Geometry: final body of the model. Coordinates: model frame, mm. Give positions to 0.01 mm unless a question says otherwise; leave off trailing zeros. Write each loop counter-clockwise with the first axis right and the second up, starting at its lowest first coordinate (ties: lowest second). Pieces come first, ordered by that corner, then holes.
Q1. Section C-C (y = 73). Return the cut outline in (x, z).
Q2. Section A-A (z = 0.65). Return the cut outline in (x, y).
Q3. Pin query (flat end, axial travel): pin 1 Ø1.5 at (y, z) = (98.5, 1.5) entering from -X; pin 2 Ø0.9 at (y, z) = (144.5, 1.5) entering from -X; pin 3 Ø10 at (x, y) = (-17, 112.5) entering from -Z; pin 4 Ø0.9 at (x, z) = (-12.5, 1.5) entering from +Y. Return the tip coordinate at first contact, or that it passes through.
Q4. Section D-D (y = 51). Return the cut outline in (x, z), plus the area to 3 significant figures.
Q5. Line query: line 1 (Y direction, x = -12, z = 2); line 2 (Y direction, x = -14.5, z = 0.45); line 3 (X direction, y = 29.5, z = 0.7). Output: solid intervals per line, ascending.
Q6. Section B-B (x = -12). Return the cut outline in (y, z), plus the area to 4 significant figures.
from build123d import *

# Parameters (mm, degrees)
SKETCH1_W           = 2.9
SKETCH1_H           = 20
BOSS_EXTRUDE1_DEPTH = 3
FILLET1_R           = 5
FILLET2_R           = 30
SKETCH4_R           = 2.3
CUT_EXTRUDE1_DEPTH  = 10
SKETCH5_W           = 20
SKETCH5_H           = 2.9
CUT_EXTRUDE2_DEPTH  = 165.164551594


with BuildPart() as part:
    # Sketch1 → Boss-Extrude1 (new body)
    with BuildSketch(Plane.XY):
        Polygon((0, 0), (-23, 0), (-23, 68), (-75, 143), (-47.5, 143), (-47.5, 146), (-27.5, 146), (-27.5, 143), (0, 143), align=None)
        with Locations((-16.5, 15)):
            Rectangle(SKETCH1_W, SKETCH1_H, mode=Mode.SUBTRACT)
        with Locations((-6.5, 15)):
            Rectangle(SKETCH1_W, SKETCH1_H, mode=Mode.SUBTRACT)
    extrude(amount=BOSS_EXTRUDE1_DEPTH)

    # Fillet1
    fillet1_edges = [part.edges().sort_by_distance(p)[0] for p in [
        (0, 0, 1.5),
        (-23, 0, 1.5),
    ]]
    fillet(fillet1_edges, radius=FILLET1_R)

    # Fillet2
    fillet2_edges = [part.edges().sort_by_distance(p)[0] for p in [
        (-23, 68, 1.5),
    ]]
    fillet(fillet2_edges, radius=FILLET2_R)

    # Sketch4 → Cut-Extrude1 (cut)
    with BuildSketch(Plane.XY.offset(3)):
        with Locations((-12, 73)):
            Circle(SKETCH4_R)
    extrude(amount=-CUT_EXTRUDE1_DEPTH, mode=Mode.SUBTRACT)

    # Sketch5 → Cut-Extrude2 (cut, through all)
    with BuildSketch(Plane(origin=(0, 0, 0), x_dir=(-1, 0, 0), z_dir=(0, 0, -1))):
        with Locations((15, 98)):
            Rectangle(SKETCH5_W, SKETCH5_H)
    extrude(amount=-CUT_EXTRUDE2_DEPTH, mode=Mode.SUBTRACT)


solid = part.part
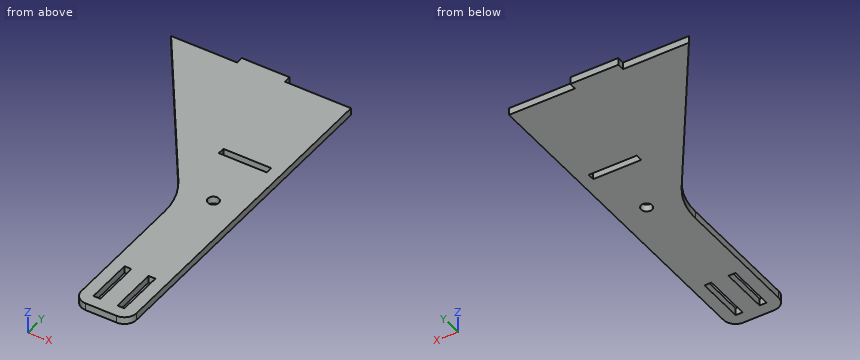
Computed:
1. outline: (-26.67, 0) - (-14.3, 0) - (-14.3, 3) - (-26.67, 3) - close; (-9.7, 0) - (0, 0) - (0, 3) - (-9.7, 3) - close
2. outline: (-75, 143) - (-28.35, 75.71) arc R30 cw to (-23, 58.62) - (-23, 5) arc R5 ccw to (-18, 0) - (-5, 0) arc R5 ccw to (0, 5) - (0, 143) - (-27.5, 143) - (-27.5, 146) - (-47.5, 146) - (-47.5, 143) - close; hole (-25, 96.55) - (-5, 96.55) - (-5, 99.45) - (-25, 99.45) - close; hole (-17.95, 5) - (-15.05, 5) - (-15.05, 25) - (-17.95, 25) - close; hole circle Ø4.6 at (-12, 73); hole (-7.95, 5) - (-5.05, 5) - (-5.05, 25) - (-7.95, 25) - close
3. pin 1: stops at x = -44.67
3. pin 2: stops at x = -47.5
3. pin 3: stops at z = 0
3. pin 4: stops at y = 143
4. outline: (-23, 0) - (0, 0) - (0, 3) - (-23, 3) - close
4. area: 69.0 mm2
5. line 1: y = 0 to 70.7, 75.3 to 96.55, 99.45 to 143
5. line 2: y = 0 to 96.55, 99.45 to 143
5. line 3: x = -23 to 0
6. outline: (0, 0) - (70.7, 0) - (70.7, 3) - (0, 3) - close; (75.3, 0) - (96.55, 0) - (96.55, 3) - (75.3, 3) - close; (99.45, 0) - (143, 0) - (143, 3) - (99.45, 3) - close
6. area: 406.5 mm2
